The figure shows three views and two pictorial views of one solid part (mm, origin at its lowest corner). Answer the questions. Round coordinates to 2 decimals unless told otherwise and drop trailing zeros. Write each loop counter-clockwise with the first axis right and the second up, starting at its lowest first coordinate (ties: lowest second). Pieces come first, ordered by that corner, then holes.
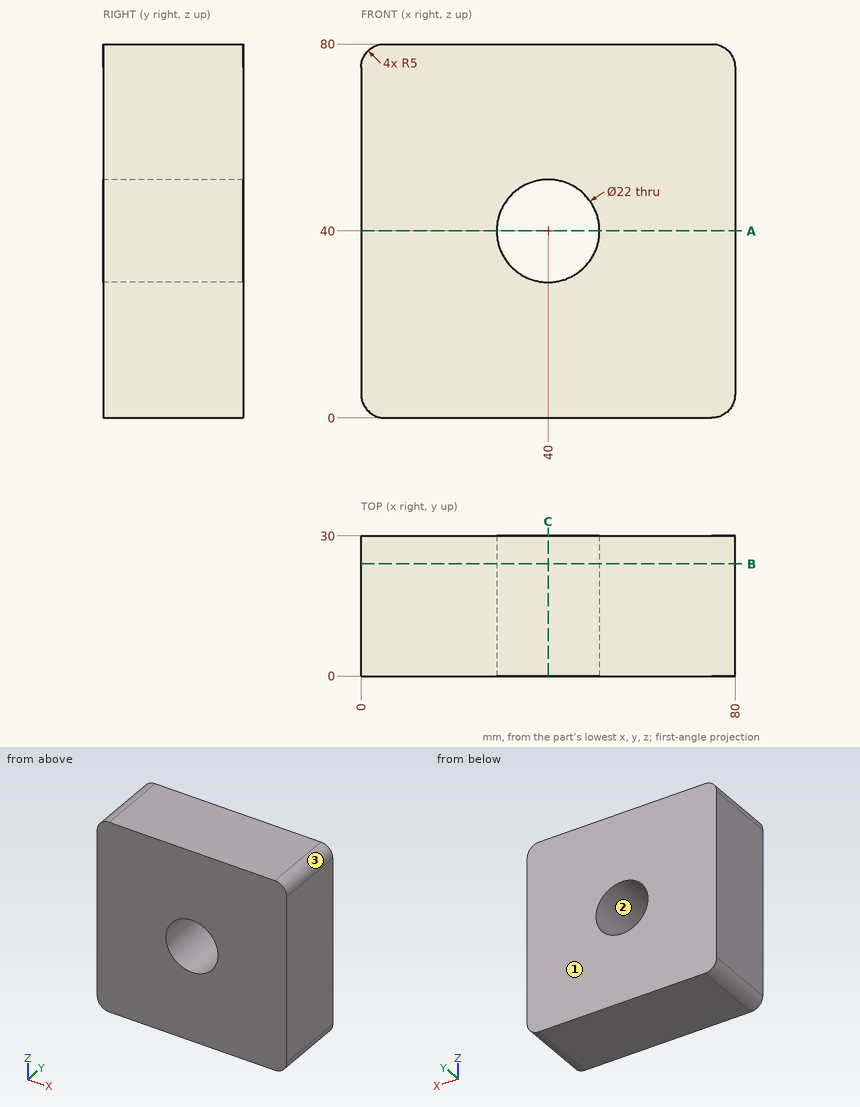
Q1. Straight lines are drawn through the part: probe 1 along Z at (x, y) = (40, 7.75); probe 2 along X at (y, z) = (1.5, 45). For each, find the intervals that lie inside material, in ascending order.
Verdict:
probe 1: z = 0 to 29, 51 to 80
probe 2: x = 0 to 30.2, 49.8 to 80
Q2. Section A-A (z = 40) is taken. Determine the outline of the cut face in (x, y).
Verdict:
outline: (0, 0) - (29, 0) - (29, 30) - (0, 30) - close; (51, 0) - (80, 0) - (80, 30) - (51, 30) - close
Q3. A flat-ended cylindrical pin translates along its axis: pin 1 Ø13 at (x, z) = (40, 40) entering from +Y. Find the tip coordinate at first contact, or state that the pin passes through.
Verdict:
pin 1: passes through
Q4. Section B-B (y = 24) is taken. Determine the outline of the cut face in (x, z).
Verdict:
outline: (0, 5) arc R5 ccw to (5, 0) - (75, 0) arc R5 ccw to (80, 5) - (80, 75) arc R5 ccw to (75, 80) - (5, 80) arc R5 ccw to (0, 75) - close; hole circle Ø22 at (40, 40)
Q5. Section C-C (x = 40) is taken. Determine the outline of the cut face in (y, z).
Verdict:
outline: (0, 0) - (30, 0) - (30, 29) - (0, 29) - close; (0, 51) - (30, 51) - (30, 80) - (0, 80) - close
Q6. Determine the mould class of the marked faces 1, 2 and 3 for opening direction X: pulls with the +X half, pulls with the -X half, needs draft (parallel to the pull), parting line crosses it, or undercut.
Verdict:
face 1: needs draft
face 2: undercut
face 3: pulls with the +X half
